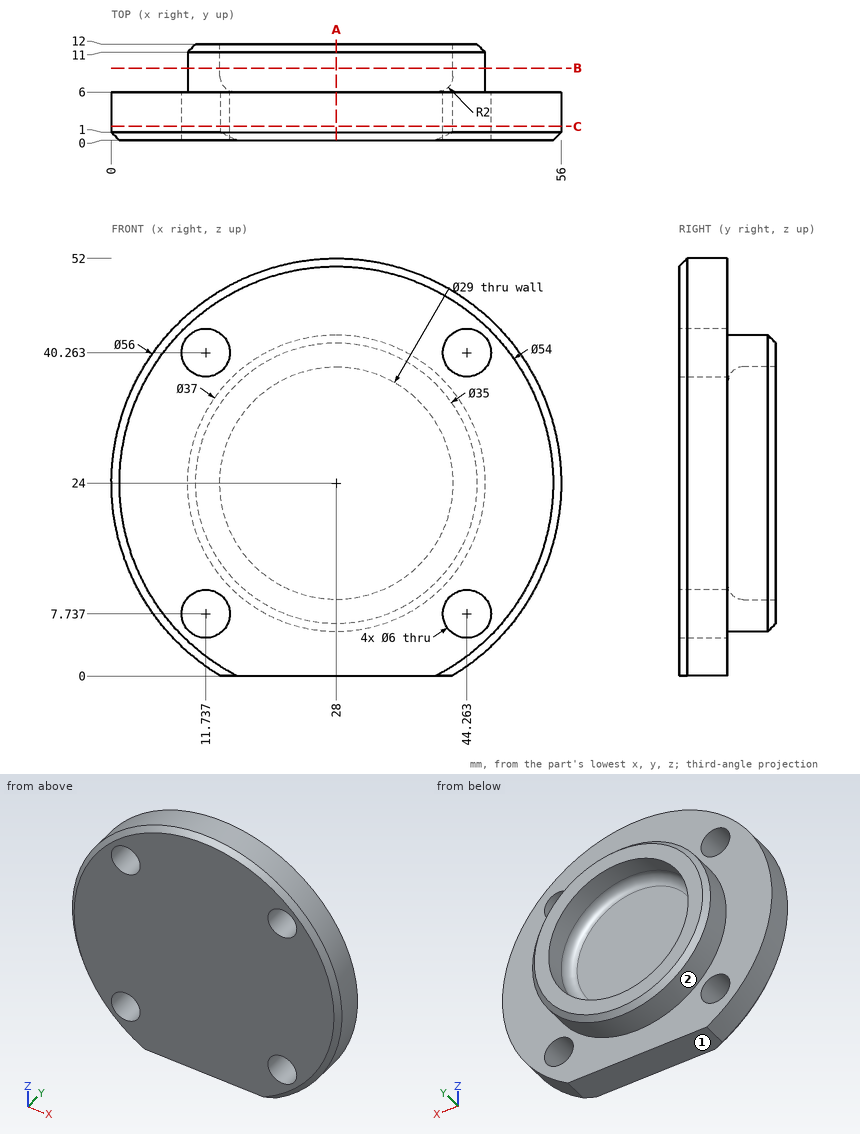
The drawing under review shows one solid part. Ordinate dimensions are in mm from its lowest x, y, z. A direction names the side the tool comes from. Round coordinates to 2 decimals unless told otherwise and drop trailing zeros. Loops run counter-clockwise (first coordinate to the right, second up) from the corner with the lowest first, then second, coordinate; pieces in that order, holes last. Notation, with made-up numbers: (4, -7.75) - (24, -7.75) arc R21 cw to (24, 26.25) - close; hole circle Ø6 at (0, 7.5). An arc over 180 degrees is marked (long way). One line per item, written item: value. Start each with the question number.
1) Insertion check: pin 1 Ø3 at (x, y) = (32, 6.5) entering from +Z; pin 2 Ø1 at (x, z) = (31, 8) entering from -Y; pin 3 Ø7 at (x, z) = (11.74, 40.26) entering from +Y; pin 4 Ø6 at (y, z) = (6.5, 28.5) entering from -X. Each pin has a flat end and moves straight along its axis. Give the tip position at first contact, or say it passes through.
2) Consider section B-B on y = 9. Give the boundary of the cut face in (x, z), then the cut area to 3 significant figures.
3) Consider section A-A on x = 28. Give the boundary of the cut face in (y, z).
4) To check wall thickness, follow L1, parallel to X at y = 1.5, z = 43 (1 decimal); L2, parallel to X at y = 11, z = 24; L3, parallel to Y at x = 31, z = 21. State the ranges of each line that lie inside material, in increasing order. Write a range as from..to.
5) For the marked faces 1 and 2, list the 3-axis set-ups (+Z, -Z, +X, -X, +Y, -Y) from which the entire face can be reached by the end or side of a thin tool; tool diameter is ignored.
6) Consider section C-C on y = 1.75. Give the boundary of the cut face in (x, z), then the cut area to 3 significant figures.
Reported:
1. pin 1: stops at z = 51.88
1. pin 2: stops at y = 0
1. pin 3: stops at y = 6
1. pin 4: stops at x = 0.04
2. outline: circle Ø37 at (28, 24); hole circle Ø29 at (28, 24)
2. area: 415 mm^2
3. outline: (0, 0) - (6, 0) - (6, 5.5) - (11, 5.5) - (12, 6.5) - (12, 9.5) - (8, 9.5) arc R2 cw to (6, 11.5) - (6, 36.5) arc R2 cw to (8, 38.5) - (12, 38.5) - (12, 41.5) - (11, 42.5) - (6, 42.5) - (6, 52) - (1, 52) - (0, 51) - close
4. L1: x = 7.4..10.5, 13..43, 45.5..48.6
4. L2: x = 9.5..13.5, 42.5..46.5
4. L3: y = 0..6
5. face 1: -Z, +X, -X, +Y, -Y
5. face 2: +Y
6. outline: (13.58, 0) - (42.42, 0) arc R28 ccw (long way) to start; hole circle Ø6 at (11.74, 7.74); hole circle Ø6 at (11.74, 40.26); hole circle Ø6 at (44.26, 7.74); hole circle Ø6 at (44.26, 40.26)
6. area: 2,270 mm^2
